Geometry: final body of the model. Coordinates: model frame, mm. Give positions to 0.01 mm unless a question says otherwise; leave off trailing zeros. Loops run counter-clockwise (first coordinate to the right, second up) from the corner with the lowest first, then second, coordinate; pieces in that order, holes last.
```python
from build123d import *

# Parameters (mm, degrees)
BOSS_EXTRUDE1_DEPTH = 11
CHAMFER1_SIZE       = 0.5


with BuildPart() as part:
    # Sketch1 → Boss-Extrude1 (new body)
    with BuildSketch(Plane.XY):
        with BuildLine():
            Line((0, 9), (28, 9))
            ThreePointArc((28, 9), (37, 0), (28, -9))
            Line((28, -9), (0, -9))
            Line((0, -9), (-28, -9))
            ThreePointArc((-28, -9), (-37, 0), (-28, 9))
            Line((-28, 9), (0, 9))
        make_face()
    extrude(amount=BOSS_EXTRUDE1_DEPTH)

    # Chamfer1
    chamfer1_edges = [part.edges().sort_by_distance(p)[0] for p in [
        (0, -9, 11),
        (37, 0, 11),
        (0, 9, 11),
        (0, 9, 0),
        (37, 0, 0),
        (0, -9, 0),
        (-37, 0, 0),
        (-37, 0, 11),
    ]]
    chamfer(chamfer1_edges, length=CHAMFER1_SIZE)


solid = part.part
```
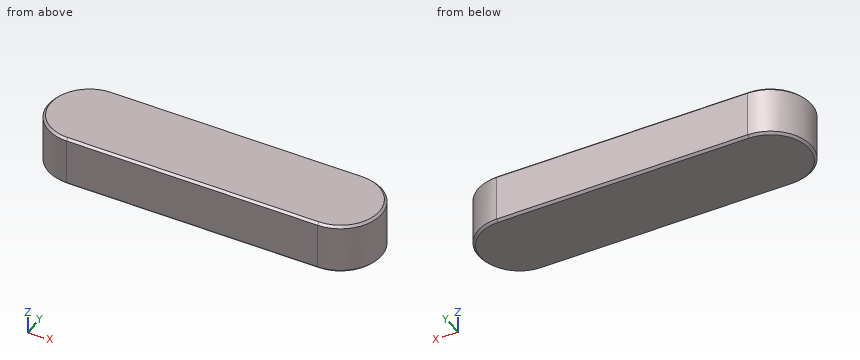
Q1. Pin query (flat end, axial travel): pin 1 Ø1 at (y, z) = (-1.5, 5.5) entering from +X; pin 2 Ø1.5 at (y, z) = (-6, 4) entering from -X; pin 3 Ø5 at (y, z) = (-7, 9.5) entering from -X. Return the tip coordinate at first contact, or that it passes through.
Q2. Section query A-A, the plane z = 1.75. Return loops of the section in (x, y).
Q3. Material intervals for probe 1 along Y at (x, z) = (31, 4); probe 2 along X at (y, z) = (-3, 8.25); probe 3 along X at (y, z) = (0.5, 3), sorted ascending.
Resolved:
1. pin 1: stops at x = 36.94
1. pin 2: stops at x = -35.31
1. pin 3: stops at x = -35.79
2. outline: (-28, -9) - (28, -9) arc R9 ccw to (28, 9) - (-28, 9) arc R9 ccw to start
3. probe 1: y = -8.49 to 8.49
3. probe 2: x = -36.49 to 36.49
3. probe 3: x = -36.99 to 36.99
